Read the model definition and answer for the solid it produces. Units are mm, in the model's axes. A direction names the side the tool comes from. Give positions to 0.01 mm unless a question says otherwise; leave off trailing zeros. Order: outer loops, then holes, each group sorted by start corner. A loop starts at its lowest first (then second) coordinate and runs counter-clockwise, first axis right, second up. Notation, with made-up numbers: (23, -16) - (80, -16) arc R28 ccw to (80, 21) - close; hole circle Ø6 at (-4.5, 4). An arc over 180 degrees is marked (long way). Return JSON: item names as keys, results as strings.
```python
from build123d import *

# Parameters (mm, degrees)
SKETCH1_R           = 75
SKETCH1_R_2         = 35
BOSS_EXTRUDE1_DEPTH = 22
BOSS_EXTRUDE2_START = 22
SKETCH2_R           = 50
SKETCH2_R_2         = 35
BOSS_EXTRUDE2_DEPTH = 50
CUT_EXTRUDE1_START  = 58.35
SKETCH3_R           = 50
SKETCH3_R_2         = 47.5
CUT_EXTRUDE1_DEPTH  = 2.65
SKETCH5_R           = 4
CUT_EXTRUDE2_DEPTH  = 129.195163715
CHAMFER1_SIZE       = 1


with BuildPart() as part:
    # Sketch1 → Boss-Extrude1 (new body)
    with BuildSketch(Plane.XY):
        Circle(SKETCH1_R)
        Circle(SKETCH1_R_2, mode=Mode.SUBTRACT)
    extrude(amount=BOSS_EXTRUDE1_DEPTH)

    # Sketch2 → Boss-Extrude2 (add)
    with BuildSketch(Plane.XY.offset(BOSS_EXTRUDE2_START)):
        Circle(SKETCH2_R)
        Circle(SKETCH2_R_2, mode=Mode.SUBTRACT)
    extrude(amount=BOSS_EXTRUDE2_DEPTH)

    # Sketch3 → Cut-Extrude1 (cut)
    with BuildSketch(Plane.XY.offset(CUT_EXTRUDE1_START)):
        Circle(SKETCH3_R)
        Circle(SKETCH3_R_2, mode=Mode.SUBTRACT)
    extrude(amount=CUT_EXTRUDE1_DEPTH, mode=Mode.SUBTRACT)

    # Sketch5 → Cut-Extrude2 (cut, through all)
    with BuildSketch(Plane(origin=(0, 0, 0), x_dir=(-1, 0, 0), z_dir=(0, 0, -1))):
        with Locations((-17.413936667, 65.732448682)):
            Circle(SKETCH5_R)
        with Locations((48.219002079, 47.947135874)):
            Circle(SKETCH5_R)
        with Locations((65.632938745, -17.785312808)):
            Circle(SKETCH5_R)
        with Locations((17.413936667, -65.732448682)):
            Circle(SKETCH5_R)
        with Locations((-48.219002079, -47.947135874)):
            Circle(SKETCH5_R)
        with Locations((-65.632938745, 17.785312808)):
            Circle(SKETCH5_R)
    extrude(amount=-CUT_EXTRUDE2_DEPTH, mode=Mode.SUBTRACT)

    # Chamfer1
    chamfer1_edges = [part.edges().sort_by_distance(p)[0] for p in [
        (21.413936667, 65.732448682, 0),
        (-44.219002079, 47.947135874, 0),
        (-61.632938745, -17.785312808, 0),
        (-13.413936667, -65.732448682, 0),
        (52.219002079, -47.947135874, 0),
        (69.632938745, 17.785312808, 0),
    ]]
    chamfer(chamfer1_edges, length=CHAMFER1_SIZE)

    # Sketch7 → Cut-Revolve1 (revolve, cut)
    with BuildSketch(Plane(origin=(0, 0, 0), x_dir=(0, 0, -1), z_dir=(1, 0, 0)), mode=Mode.PRIVATE) as cut_revolve1_sk:
        Polygon((-72, 35), (-72, 36.5), (-70, 37.654700538), (-70, 40), (-65.7, 40), (-65.7, 35), align=None)
    revolve(cut_revolve1_sk.sketch.rotate(Axis((0, 0, 72), (0, 0, -1)), 90), axis=Axis((0, 0, 72), (0, 0, -1)), mode=Mode.SUBTRACT)


solid = part.part
```
Q1. A cutting plane is placed at A-A (y = 0). Write down the section's boundary in (x, z), and give its area (3 significant figures).
Values:
{"outline": "(-75, 0) - (-35, 0) - (-35, 65.7) - (-40, 65.7) - (-40, 70) - (-37.65, 70) - (-36.5, 72) - (-50, 72) - (-50, 61) - (-47.5, 61) - (-47.5, 58.35) - (-50, 58.35) - (-50, 22) - (-75, 22) - close; (35, 0) - (75, 0) - (75, 22) - (50, 22) - (50, 58.35) - (47.5, 58.35) - (47.5, 61) - (50, 61) - (50, 72) - (36.5, 72) - (37.65, 70) - (40, 70) - (40, 65.7) - (35, 65.7) - close", "area": "3,200 mm²"}
Q2. A cutting plane is placed at D-D (x = 17.5). Give the number of separate pieces and of enclosed holes in the cut face, and give its area (3 significant figures).
Values:
{"separate pieces": "3", "enclosed holes": "0", "area": "3,280 mm²"}
Q3. Given pin 1 (5 mm diameter, centred on x = 27.5, z = 52, fed in from -Y); pin 2 (5 mm diameter, centred on y = 26.5, z = 57, fed in from -X); pin 3 (1.5 mm diameter, centred on x = 46.5, y = 2.5, fed in from -Z); pin 4 (3 mm diameter, centred on y = -60, z = 7.5, fed in from -X), each flat-ended and moving along its own axis, determine where each tip first touches the part or whether it passes through.
Values:
{"pin 1": "stops at y = -43.3", "pin 2": "stops at x = -43.86", "pin 3": "stops at z = 0", "pin 4": "stops at x = -46.93"}
Q4. Consider L1, parallel to Z at x = -46, y = -16.5; L2, parallel to Y at x = -18, z = 9.5; L3, parallel to Y at x = 0, z = 66. Determine where each line is inside the solid, lowest interval first.
Values:
{"L1": "z = 0 to 58.35, 61 to 72", "L2": "y = -72.81 to -69.69, -61.78 to -30.02, 30.02 to 72.81", "L3": "y = -50 to -40, 40 to 50"}
Q5. A cutting plane is placed at C-C (z = 30.5). Write down the section's boundary in (x, y).
Values:
{"outline": "circle Ø100 at (0, 0); hole circle Ø70 at (0, 0)"}
Q6. Determine the mould class of faces 1 (the cylindrical face through (-10.3, -46.37, 59.66)), 2 (the flat face through (32, -16, 0)), 3 (the flat face through (3, -37, 72)), 4 (the cylindrical face through (47.69, 15.02, 39.92)) for opening direction Z: released by +Z, released by -Z, zero draft, split by the parting line, or undercut.
Values:
{"face 1": "undercut", "face 2": "released by -Z", "face 3": "released by +Z", "face 4": "zero draft"}
Q7. For faces 5 (the cylindrical face through (-45.045, 45.513, 11.353)), 6 (the cylindrical face through (47.69, 15.02, 66.42)), 7 (the flat face through (44.2, -18.3, 61)), determine the directions among +Z, -Z, +X, -X, +Y, -Y from which every point of the face is accessible in a straight line to the end or side of a thin tool.
Values:
{"face 5": "+Z, -Z", "face 6": "+Z", "face 7": "none"}
